from build123d import *

# Parameters (mm, degrees)
SKETCH_1_W                = 40
SKETCH_1_H                = 80
EXTRUDE_1_DEPTH           = 2
HOLE_WIZARD_1_D           = 9
HOLE_WIZARD_1_DEPTH       = 10
HOLE_WIZARD_1_CSINK_D     = 17.3
HOLE_WIZARD_1_CSINK_ANGLE = 90
HOLE_WIZARD_1_TIP         = 2.703872786
CHAMFER_1_SIZE            = 1


with BuildPart() as part:
    # 草图1 → 凸台-拉伸1 (new, symmetric)
    with BuildSketch(Plane.XY):
        Rectangle(SKETCH_1_W, SKETCH_1_H)
    extrude(amount=EXTRUDE_1_DEPTH, both=True)

    # 打孔尺寸(%根据十字)槽沉头木螺钉的类型1
    with Locations(Plane(origin=(0, 20, 2), x_dir=(1, 0, 0), z_dir=(0, 0, 1))):
        with Locations((0, 0), (0, -40)):
            CounterSinkHole(HOLE_WIZARD_1_D / 2, HOLE_WIZARD_1_CSINK_D / 2, depth=HOLE_WIZARD_1_DEPTH, counter_sink_angle=HOLE_WIZARD_1_CSINK_ANGLE)
            with Locations((0, 0, -(HOLE_WIZARD_1_DEPTH + HOLE_WIZARD_1_TIP / 2))):  # 118° drill point
                Cone(0, HOLE_WIZARD_1_D / 2, HOLE_WIZARD_1_TIP, mode=Mode.SUBTRACT)

    # 倒角1
    chamfer_1_edges = [part.edges().sort_by_distance(p)[0] for p in [
        (-20, 0, 2),
        (0, -40, 2),
        (20, 0, 2),
        (0, 40, 2),
    ]]
    chamfer(chamfer_1_edges, length=CHAMFER_1_SIZE)


solid = part.part
The model under review builds one solid part; all positions refer to its coordinate system, in mm. Coordinates: 2 decimals unless noted, no trailing zeros. Write each loop counter-clockwise with the first axis right and the second up, starting at its lowest first coordinate (ties: lowest second). Pieces come first, ordered by that corner, then holes. Notation, with made-up numbers: (-37.75, 4.5) - (-26.75, 4.5) arc R13 cw to (-26.75, 20.5) - close; hole circle Ø1 at (15, 62.25). An arc over 180 degrees is marked (long way). Answer as CSV lines item,"result".
(1) We need section A-A (x = 0). Give the boundary of the cut face in (y, z).
Data:
outline,"(-40, -2) - (-24.65, -2) - (-28.65, 2) - (-39, 2) - (-40, 1) - close; (-15.35, -2) - (15.35, -2) - (11.35, 2) - (-11.35, 2) - close; (24.65, -2) - (40, -2) - (40, 1) - (39, 2) - (28.65, 2) - close"
(2) For line 1 along Y through (x, z) = (-5.5, 1.75); line 2 along Y through (x, z) = (2, -1.3); line 3 along X through (y, z) = (-19.5, 1.25), list the stretches that pass through material, from the lowest coordinate up. Write a range as [from, to].
Data:
line 1,"y = [-39.25, -26.35], [-13.65, 13.65], [26.35, 39.25]"
line 2,"y = [-40, -24.96], [-15.04, 15.04], [24.96, 40]"
line 3,"x = [-19.75, -7.88], [7.88, 19.75]"
(3) We need section B-B (z = -1.35). Give the boundary of the cut face in (x, y), plus the area to 3 significant figures.
Data:
outline,"(-20, -40) - (20, -40) - (20, 40) - (-20, 40) - close; hole circle Ø10.6 at (0, -20); hole circle Ø10.6 at (0, 20)"
area,"3,020 mm2"
(4) Mouldability with a two-part tool opening along Y and no side actions: class faces 1 (the conical face through (0.63, -15.2, -1.81)), 2 (the flat face through (0, 40, 0)), 3 (the flat face through (0, 1, 2)) as pulls with the +Y half, pulls with the -Y half, needs draft (parallel to the pull), parting line crosses it, or undercut.
Data:
face 1,"undercut"
face 2,"pulls with the +Y half"
face 3,"needs draft"
(5) We need section C-C (y = 20). Give the boundary of the cut face in (x, z), plus the area to 3 significant figures.
Data:
outline,"(-20, -2) - (-4.65, -2) - (-8.65, 2) - (-19, 2) - (-20, 1) - close; (4.65, -2) - (20, -2) - (20, 1) - (19, 2) - (8.65, 2) - close"
area,"106 mm2"
